from build123d import *

# Parameters (mm, degrees)
SKETCH1_W           = 50
SKETCH1_H           = 50
SKETCH1_W_2         = 46
SKETCH1_H_2         = 46
BOSS_EXTRUDE1_DEPTH = 600
SKETCH2_R           = 5.5
CUT_EXTRUDE1_DEPTH  = 50


with BuildPart() as part:
    # Sketch1 → Boss-Extrude1 (new body)
    with BuildSketch(Plane.XY):
        Rectangle(SKETCH1_W, SKETCH1_H)
        Rectangle(SKETCH1_W_2, SKETCH1_H_2, mode=Mode.SUBTRACT)
    extrude(amount=BOSS_EXTRUDE1_DEPTH)

    # Sketch2 → Cut-Extrude1 (cut)
    with BuildSketch(Plane(origin=(0, 25, 0), x_dir=(1, 0, 0), z_dir=(0, 1, 0))):
        with Locations(Location((0, -225, 0), (0, 0, 270))):
            Circle(SKETCH2_R)
        with Locations(Location((0, -375, 0), (0, 0, 270))):
            Circle(SKETCH2_R)
    extrude(amount=-CUT_EXTRUDE1_DEPTH, mode=Mode.SUBTRACT)


solid = part.part
Read the model definition and answer for the solid it produces. Units are mm, in the model's axes. A direction names the side the tool comes from. Give positions to 0.01 mm unless a question says otherwise; leave off trailing zeros. Loops run counter-clockwise (first coordinate to the right, second up) from the corner with the lowest first, then second, coordinate; pieces in that order, holes last. Notation, with made-up numbers: (-39, 24) -> (-8, 24) arc R15 ccw to (-8, 40) -> close; hole circle Ø11 at (4, -27.5). An arc over 180 degrees is marked (long way). Use a Markdown table: item, result.
Q1. Section C-C, the plane y = 8 is taken. Determine the outline of the cut face in (x, z), then the cut area to 3 significant figures.
Solved:
| item | result |
|---|---|
| outline | (-25, 0) -> (-23, 0) -> (-23, 600) -> (-25, 600) -> close; (23, 0) -> (25, 0) -> (25, 600) -> (23, 600) -> close |
| area | 2,400 mm^2 |
Q2. Determine the mould class of faces 1 (the face through (0, -23, 296)), 2 (the face through (25, 0, 296)), 3 (the face through (-2, -24, 0)) for opening direction X: pulls with the +X half, pulls with the -X half, needs draft (parallel to the pull), parting line crosses it, or undercut.
Solved:
| item | result |
|---|---|
| face 1 | undercut |
| face 2 | pulls with the +X half |
| face 3 | needs draft |
Q3. Section D-D, the plane z = 375 is taken. Determine the outline of the cut face in (x, y).
Solved:
| item | result |
|---|---|
| outline | (-25, -25) -> (-5.5, -25) -> (-5.5, -23) -> (-23, -23) -> (-23, 23) -> (-5.5, 23) -> (-5.5, 25) -> (-25, 25) -> close; (5.5, -25) -> (25, -25) -> (25, 25) -> (5.5, 25) -> (5.5, 23) -> (23, 23) -> (23, -23) -> (5.5, -23) -> close |
Q4. A tool of negligible diameter and unlimited length cuts with its end or side. For faces 4 (the face through (0, -25, 296)), 5 (the face through (0, 23, 296)), from which of +Z, -Z, +X, -X, +Y, -Y can it reach the whole face along a straight path? Write none if from no direction.
Solved:
| item | result |
|---|---|
| face 4 | +Z, -Z, +X, -X, -Y |
| face 5 | +Z, -Z |
Q5. Find the intervals of material crossed by line 1 along Y through (x, z) = (13.5, 129.5); line 2 along X through (y, z) = (24.6, 225), in increasing order.
Solved:
| item | result |
|---|---|
| line 1 | y = -25 to -23, 23 to 25 |
| line 2 | x = -25 to -5.5, 5.5 to 25 |
Q6. Section B-B, the plane x = 0 is taken. Determine the outline of the cut face in (y, z), then the cut area to 3 significant figures.
Solved:
| item | result |
|---|---|
| outline | (-25, 0) -> (-23, 0) -> (-23, 219.5) -> (-25, 219.5) -> close; (-25, 230.5) -> (-23, 230.5) -> (-23, 369.5) -> (-25, 369.5) -> close; (-25, 380.5) -> (-23, 380.5) -> (-23, 600) -> (-25, 600) -> close; (23, 0) -> (25, 0) -> (25, 219.5) -> (23, 219.5) -> close; (23, 230.5) -> (25, 230.5) -> (25, 369.5) -> (23, 369.5) -> close; (23, 380.5) -> (25, 380.5) -> (25, 600) -> (23, 600) -> close |
| area | 2,310 mm^2 |
Q7. Section A-A, the plane z = 110 is taken. Determine the outline of the cut face in (x, y), then the cut area to 3 significant figures.
Solved:
| item | result |
|---|---|
| outline | (-25, -25) -> (25, -25) -> (25, 25) -> (-25, 25) -> close; hole (-23, -23) -> (23, -23) -> (23, 23) -> (-23, 23) -> close |
| area | 384 mm^2 |
